```python
from build123d import *

# Parameters (mm, degrees)
BOSS_EXTRUDE1_DEPTH = 6
SKETCH2_R           = 4
CUT_EXTRUDE1_DEPTH  = 95


with BuildPart() as part:
    # Sketch1 → Boss-Extrude1 (new body)
    with BuildSketch(Plane.XY):
        with BuildLine():
            Line((0, 10), (57.02, 10))
            ThreePointArc((57.02, 10), (67.02, 0), (57.02, -10))
            Line((57.02, -10), (0, -10))
            ThreePointArc((0, -10), (-10, 0), (0, 10))
        make_face()
    extrude(amount=BOSS_EXTRUDE1_DEPTH)

    # Sketch2 → Cut-Extrude1 (cut)
    with BuildSketch(Plane.XY.offset(6)):
        Circle(SKETCH2_R)
        with Locations((57.02, 0)):
            Circle(SKETCH2_R)
    extrude(amount=-CUT_EXTRUDE1_DEPTH, mode=Mode.SUBTRACT)


solid = part.part
```
For this review, take the finished solid that the model builds, in its own axes (mm). Round coordinates to 2 decimals unless told otherwise and drop trailing zeros. Order: outer loops, then holes, each group sorted by start corner. A loop starts at its lowest first (then second) coordinate and runs counter-clockwise, first axis right, second up. Notation, with made-up numbers: (4.5, 5.5) -> (12.5, 5.5) arc R5 ccw to (12.5, 11.5) -> close; hole circle Ø4 at (69.25, 83.25). An arc over 180 degrees is marked (long way). Use a Markdown table: item, result.
Item 1: Draft analysis for pull direction Y (two halves, no side actions). For faces 1 (the flat face through (29, -10, 3)), 2 (the cylindrical face through (-0.867, -3.905, 3.042)), 3 (the cylindrical face through (-10, 0, 3)), state which applies: +Y half, -Y half, draft (parallel to the pull), parting line (faces both ways), or undercut.
Resolved:
| item | result |
|---|---|
| face 1 | -Y half |
| face 2 | undercut |
| face 3 | parting line |
Item 2: Take a section at A-A (y = 0). State the section outline as (x, z) points.
Resolved:
| item | result |
|---|---|
| outline | (-10, 0) -> (-4, 0) -> (-4, 6) -> (-10, 6) -> close; (4, 0) -> (53.02, 0) -> (53.02, 6) -> (4, 6) -> close; (61.02, 0) -> (67.02, 0) -> (67.02, 6) -> (61.02, 6) -> close |
Item 3: Take a section at D-D (y = -6.75). State the section outline as (x, z) points, plus the area to 3 significant figures.
Resolved:
| item | result |
|---|---|
| outline | (-7.38, 0) -> (64.4, 0) -> (64.4, 6) -> (-7.38, 6) -> close |
| area | 431 mm² |
Item 4: Take a section at B-B (z = 4). State the section outline as (x, y) points, plus the area to 3 significant figures.
Resolved:
| item | result |
|---|---|
| outline | (0, -10) -> (57.02, -10) arc R10 ccw to (57.02, 10) -> (0, 10) arc R10 ccw to start; hole circle Ø8 at (0, 0); hole circle Ø8 at (57.02, 0) |
| area | 1,350 mm² |
Item 5: For pin 1 (1 mm diameter, centred on y = -3, z = 3.5, fed in from -X), flat-tipped, find the tip position at first contact; note if it passes through.
Resolved:
| item | result |
|---|---|
| pin 1 | stops at x = -9.68 |
Item 6: For line 1 along Y through (x, z) = (0, 2.2); line 2 along X through (y, z) = (1.5, 0.85); line 3 along X through (y, z) = (0.5, 2.65), list the stretches that pass through material, from the lowest coordinate up. Write a range as [from, to].
Resolved:
| item | result |
|---|---|
| line 1 | y = [-10, -4], [4, 10] |
| line 2 | x = [-9.89, -3.71], [3.71, 53.31], [60.73, 66.91] |
| line 3 | x = [-9.99, -3.97], [3.97, 53.05], [60.99, 67.01] |
Item 7: Take a section at C-C (x = 60). State the section outline as (y, z) points, plus the area to 3 significant figures.
Resolved:
| item | result |
|---|---|
| outline | (-9.55, 0) -> (-2.67, 0) -> (-2.67, 6) -> (-9.55, 6) -> close; (2.67, 0) -> (9.55, 0) -> (9.55, 6) -> (2.67, 6) -> close |
| area | 82.5 mm² |
